Read the model definition and answer for the solid it produces. Units are mm, in the model's axes. A direction names the side the tool comes from. Round coordinates to 2 decimals unless told otherwise and drop trailing zeros. Order: outer loops, then holes, each group sorted by start corner. A loop starts at its lowest first (then second) coordinate and runs counter-clockwise, first axis right, second up.
from build123d import *

# Parameters (mm, degrees)
SKETCH_1_W          = 30
SKETCH_1_H          = 30
EXTRUDE_1_DEPTH     = 415
SHELL_1_T           = -1
SKETCH_2_R          = 2.6
SKETCH_2_R_2        = 2.05
CUT_EXTRUDE_1_DEPTH = 417.353215431
SKETCH_3_R          = 7.5
CUT_EXTRUDE_2_DEPTH = 417.353215431
SKETCH_4_R          = 7.5
CUT_EXTRUDE_3_DEPTH = 417.353215431


with BuildPart() as part:
    # 草图1 → 凸台-拉伸1 (new body)
    with BuildSketch(Plane.XY):
        Rectangle(SKETCH_1_W, SKETCH_1_H)
    extrude(amount=EXTRUDE_1_DEPTH)

    # 抽壳1
    shell_1_openings = [part.faces().sort_by_distance(p)[0] for p in [
        (0, 0, 415),
        (0, 0, 0),
    ]]
    offset(amount=SHELL_1_T, openings=shell_1_openings, kind=Kind.INTERSECTION)

    # 草图2 → 切除-拉伸1 (cut, through all)
    with BuildSketch(Plane(origin=(0, 15, 0), x_dir=(1, 0, 0), z_dir=(0, 1, 0))):
        with Locations(Location((0, -159.5, 0), (0, 0, 270))):
            Circle(SKETCH_2_R)
        with Locations(Location((0, -255.5, 0), (0, 0, 270))):
            Circle(SKETCH_2_R)
        with Locations(Location((0, -207.5, 0), (0, 0, 270))):
            Circle(SKETCH_2_R)
        with Locations(Location((-10, -35, 0), (0, 0, 270))):
            Circle(SKETCH_2_R_2)
        with Locations(Location((-10, -380, 0), (0, 0, 90))):
            Circle(SKETCH_2_R_2)
        with Locations(Location((-10, -65, 0), (0, 0, 270))):
            Circle(SKETCH_2_R_2)
        with Locations(Location((-10, -350, 0), (0, 0, 90))):
            Circle(SKETCH_2_R_2)
        with Locations(Location((10, -65, 0), (0, 0, 270))):
            Circle(SKETCH_2_R_2)
        with Locations(Location((10, -350, 0), (0, 0, 90))):
            Circle(SKETCH_2_R_2)
        with Locations(Location((10, -35, 0), (0, 0, 270))):
            Circle(SKETCH_2_R_2)
        with Locations(Location((10, -380, 0), (0, 0, 90))):
            Circle(SKETCH_2_R_2)
    extrude(amount=-CUT_EXTRUDE_1_DEPTH, mode=Mode.SUBTRACT)

    # 草图3 → 切除-拉伸2 (cut, through all)
    with BuildSketch(Plane.ZY.offset(15)):
        with Locations((85.5, 0)):
            Circle(SKETCH_3_R)
        with Locations((115.5, 0)):
            Circle(SKETCH_3_R)
        with Locations((145.5, 0)):
            Circle(SKETCH_3_R)
        with Locations((269.5, 0)):
            Circle(SKETCH_3_R)
        with Locations((299.5, 0)):
            Circle(SKETCH_3_R)
        with Locations((329.5, 0)):
            Circle(SKETCH_3_R)
        with Locations((183.5, 0)):
            Circle(SKETCH_3_R)
        with Locations((231.5, 0)):
            Circle(SKETCH_3_R)
    extrude(amount=-CUT_EXTRUDE_2_DEPTH, mode=Mode.SUBTRACT)

    # 草图4 → 切除-拉伸3 (cut, through all)
    with BuildSketch(Plane(origin=(0, 15, 0), x_dir=(1, 0, 0), z_dir=(0, 1, 0))):
        with Locations(Location((0, -15, 0), (0, 0, 270))):
            Circle(SKETCH_4_R)
        with Locations(Location((0, -400, 0), (0, 0, 90))):
            Circle(SKETCH_4_R)
    extrude(amount=-CUT_EXTRUDE_3_DEPTH, mode=Mode.SUBTRACT)


solid = part.part
Q1. Straight lines are drawn through the part: probe 1 along X at (y, z) = (-14.6, 380); probe 2 along Y at (x, z) = (-4.25, 379). For each, find the intervals that lie inside material, in ascending order.
Outcome:
probe 1: x = -15 to -12.05, -7.95 to 7.95, 12.05 to 15
probe 2: y = -15 to -14, 14 to 15
Q2. A flat-ended cylindrical pin translates along its axis: pin 1 (3 mm diameter, centred on x = 0, z = 207.5, fed in from +Y). Find the tip coordinate at first contact, or state that the pin passes through.
Outcome:
pin 1: passes through
Q3. A cutting plane is placed at A-A, the plane z = 115.5. Give the vertices of the cut face in (x, y).
Outcome:
outline: (-15, -15) - (15, -15) - (15, -7.5) - (14, -7.5) - (14, -14) - (-14, -14) - (-14, -7.5) - (-15, -7.5) - close; (-15, 7.5) - (-14, 7.5) - (-14, 14) - (14, 14) - (14, 7.5) - (15, 7.5) - (15, 15) - (-15, 15) - close
Q4. For a pull along Z with two mould halves and no side action, classify faces 3 (the face through (-14.51, -2.87, 152.43)), 4 (the face through (-0.2, 15, 204.6)), 5 (the face through (-1.2, -14.4, 0)), 6 (the face through (-14.5, 5.1, 294)) as released by +Z, released by -Z, zero draft, split by the parting line, or undercut.
Outcome:
face 3: undercut
face 4: zero draft
face 5: released by -Z
face 6: undercut
Q5. A cutting plane is placed at B-B, the plane z = 166. Give the vertices of the cut face in (x, y).
Outcome:
outline: (-15, -15) - (15, -15) - (15, 15) - (-15, 15) - close; hole (-14, -14) - (14, -14) - (14, 14) - (-14, 14) - close
Q6. A cutting plane is placed at C-C, the plane z = 303. Give the vertices of the cut face in (x, y).
Outcome:
outline: (-15, -15) - (15, -15) - (15, -6.63) - (14, -6.63) - (14, -14) - (-14, -14) - (-14, -6.63) - (-15, -6.63) - close; (-15, 6.63) - (-14, 6.63) - (-14, 14) - (14, 14) - (14, 6.63) - (15, 6.63) - (15, 15) - (-15, 15) - close
Q7. For faces 1 (the face through (-14.507, 0.33, 224.007)), 2 (the face through (-14, 0, 205)), determine the directions among +Z, -Z, +X, -X, +Y, -Y from which every point of the face is accessible in a straight line to the end or side of a thin tool.
Outcome:
face 1: +X, -X
face 2: +Z, -Z
